from build123d import *

# Parameters (mm, degrees)
SKETCH1_R                       = 146.05
SKETCH1_R_2                     = 112.776
BOSS_EXTRUDE1_DEPTH             = 0.1778
F_13_16_0_8125_DIAMETER_HOLE1_D = 20.6375
F_13_16_0_8125_DIAMETER_HOLE2_D = 20.6375


with BuildPart() as part:
    # Sketch1 → Boss-Extrude1 (new body)
    with BuildSketch(Plane(origin=(0, 0, 0), x_dir=(1, 0, 0), z_dir=(0, 1, 0))):
        with Locations(Location((0, 0, 0), (0, 0, 270))):
            Circle(SKETCH1_R)
        with Locations(Location((0, 0, 0), (0, 0, 270))):
            Circle(SKETCH1_R_2, mode=Mode.SUBTRACT)
    extrude(amount=BOSS_EXTRUDE1_DEPTH)

    # 13/16 (0.8125) Diameter Hole1 (through all)
    with Locations(Plane(origin=(0, 0.1778, 0), x_dir=(1, 0, 0), z_dir=(0, 1, 0))):
        with Locations((0, 127)):
            Hole(F_13_16_0_8125_DIAMETER_HOLE1_D / 2)

    # 13/16 (0.8125) Diameter Hole2 (through all)
    with Locations(Plane(origin=(0, 0, 0), x_dir=(-1, 0, 0), z_dir=(0, -1, 0))):
        with Locations((-63.5, -109.982), (-120.77, 39.243), (-127, 0)):
            f_13_16_0_8125_diameter_hole2 = Hole(F_13_16_0_8125_DIAMETER_HOLE2_D / 2)

    # Mirror1: 13/16 (0.8125) Diameter Hole2 across plane
    add(f_13_16_0_8125_diameter_hole2.mirror(Plane(origin=(0, 0, 0), x_dir=(0, 0, 1), z_dir=(1, 0, 0))), mode=Mode.SUBTRACT)


solid = part.part
For this review, take the finished solid that the model builds, in its own axes (mm). Give positions to 0.01 mm unless a question says otherwise; leave off trailing zeros. Loops run counter-clockwise (first coordinate to the right, second up) from the corner with the lowest first, then second, coordinate; pieces in that order, holes last. Notation, with made-up numbers: M -25,-37.75 L 7,-37.75 A27 cw 7,-18.75 Z; hole C 33.25,43.5 d4. An arc over 180 degrees is marked long. Answer as a JSON object with one key per item and string values. Group by question number.
Q1. Add section C-C on z = -90. Give the boundary of the cut face in (x, y), and give its area (3 significant figures).
Q2. Add section A-A on x = 0. Give the boundary of the cut face in (y, z), and give its area (3 significant figures).
Q3. For probe 1 along Z at (x, y) = (63.5, 0.1); probe 2 along X at (y, z) = (0.1, 4); probe 3 along Z at (x, y) = (-113, 0.1), list the stretches that pass through material, from the lowest coordinate up. Write a range as [from, to].
Q4. Insertion check: P1, Ø12.5, axis at x = 120.77, z = -39.243, coming from the +Y side. The pin has a flat end and moves straight along its axis. Give the tip position at first contact, or say it passes through.
Q5. Add section B-B on z = 0. Give the boundary of the cut face in (x, y), and give its area (3 significant figures).
Q6. Add section D-D on y = 0.05. Give the number of separate pieces and of enclosed holes in the cut face, and give its area (3 significant figures).
Checked values:
{
 "1": {"outline": "M -115.02,0 L -67.96,0 L -67.96,0.18 L -115.02,0.18 Z; M 67.96,0 L 115.02,0 L 115.02,0.18 L 67.96,0.18 Z", "area": "16.7 mm²"},
 "2": {"outline": "M 0,-146.05 L 0.18,-146.05 L 0.18,-137.32 L 0,-137.32 Z; M 0,-116.68 L 0.18,-116.68 L 0.18,-112.78 L 0,-112.78 Z; M 0,112.78 L 0.18,112.78 L 0.18,146.05 L 0,146.05 Z", "area": "8.16 mm²"},
 "3": {"probe 1": "[-131.52, -93.2], [93.2, 99.66], [120.3, 131.52]", "probe 2": "[-146, -136.51], [-117.49, -112.71], [112.71, 117.49], [136.51, 146]", "probe 3": "[-92.53, -46.03], [-32.45, 92.53]"},
 "4": {"P1": "through"},
 "5": {"outline": "M -146.05,0 L -137.32,0 L -137.32,0.18 L -146.05,0.18 Z; M -116.68,0 L -112.78,0 L -112.78,0.18 L -116.68,0.18 Z; M 112.78,0 L 116.68,0 L 116.68,0.18 L 112.78,0.18 Z; M 137.32,0 L 146.05,0 L 146.05,0.18 L 137.32,0.18 Z", "area": "4.49 mm²"},
 "6": {"separate pieces": "1", "enclosed holes": "8", "area": "24,700 mm²"}
}
